CAD build for the part. Positions are in the model's coordinates, mm. Round coordinates to 2 decimals unless told otherwise and drop trailing zeros. Write each loop counter-clockwise with the first axis right and the second up, starting at its lowest first coordinate (ties: lowest second). Pieces come first, ordered by that corner, then holes. Notation, with made-up numbers: (17, 12.25) - (51, 12.25) arc R31 ccw to (51, 46.25) - close; hole circle Ø4 at (-36.5, 80.5). An arc over 180 degrees is marked (long way). Put each result on its own line as item: value. Start each with the question number.
Item 1: Cut at C-C (x = -51). Give the cut face in (y, z), and give its area (3 significant figures).
Item 2: Cut at A-A (z = 0.95). Count the separate pieces of the cut face and the enclosed holes in it, and give its area (3 significant figures).
Item 3: Pin check, flat tips, straight feed: pin 1 Ø2.5 at (x, y) = (-26.62, -9.74) entering from +Z; pin 2 Ø1.5 at (y, z) = (-11.5, 1.5) entering from -X; pin 3 Ø1.5 at (x, z) = (42.5, 1) entering from +Y; pin 4 Ø1.5 at (x, z) = (25.5, 1) entering from -Y. Stop position of each tip, or through.
Item 4: Drill centre lines: line 1 (X direction, y = -13, z = 2.85); line 2 (Y direction, x = 41.5, z = 0.6); line 3 (Y direction, x = -22.5, z = 0.55). Where is each one in solid material? Low to high. Write a range as from..to.
Item 5: Cut at B-B (x = 39.5). Give the cut face in (y, z).
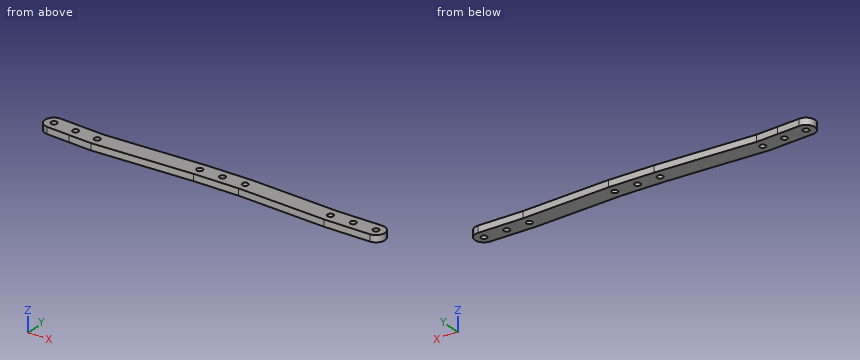
```python
from build123d import *

# Parameters (mm, degrees)
SKETCH3_R           = 1.3
SKETCH3_R_2         = 1.299999997
SKETCH3_R_3         = 1.299999994
SKETCH3_R_4         = 1.299999992
BOSS_EXTRUDE4_DEPTH = 3


with BuildPart() as part:
    # Sketch3 → Boss-Extrude4 (new body)
    with BuildSketch(Plane.XY):
        with BuildLine():
            Line((52.490961286, -7.932397294), (42.490961286, -7.932397294))
            Line((42.490961286, -7.932397294), (32.603090799, -7.932397294))
            Line((32.603090799, -7.932397294), (-6.503485734, -5.738172333))
            Line((-6.503485734, -5.738172333), (-16.615615248, -5.738172333))
            Line((-16.615615248, -5.738172333), (-26.685781884, -5.738172333))
            Line((-26.685781884, -5.738172333), (-70.669528111, -7.281743071))
            Line((-70.669528111, -7.281743071), (-80.441339321, -6.619135373))
            Line((-80.441339321, -6.619135373), (-90.418428622, -5.942608164))
            ThreePointArc((-90.418428622, -5.942608164), (-94.679875227, -9.662833001), (-90.95965039, -13.924279606))
            Line((-90.95965039, -13.924279606), (-80.982561088, -14.600806815))
            Line((-80.982561088, -14.600806815), (-70.800193694, -15.291253536))
            Line((-70.800193694, -15.291253536), (-26.545448611, -13.738172333))
            Line((-26.545448611, -13.738172333), (-16.615615248, -13.738172333))
            Line((-16.615615248, -13.738172333), (-6.727744762, -13.738172333))
            Line((-6.727744762, -13.738172333), (32.378831772, -15.932397294))
            Line((32.378831772, -15.932397294), (42.490961286, -15.932397294))
            Line((42.490961286, -15.932397294), (52.490961286, -15.932397294))
            ThreePointArc((52.490961286, -15.932397294), (56.490961286, -11.932397294), (52.490961286, -7.932397294))
        make_face()
        with Locations((-90.689039506, -9.933443885)):
            Circle(SKETCH3_R, mode=Mode.SUBTRACT)
        with Locations((-70.734860903, -11.286498303)):
            Circle(SKETCH3_R, mode=Mode.SUBTRACT)
        with Locations((-80.711950204, -10.609971094)):
            Circle(SKETCH3_R, mode=Mode.SUBTRACT)
        with Locations((-26.615615248, -9.738172333)):
            Circle(SKETCH3_R, mode=Mode.SUBTRACT)
        with Locations((-16.615615248, -9.738172333)):
            Circle(SKETCH3_R_2, mode=Mode.SUBTRACT)
        with Locations((-6.615615248, -9.738172333)):
            Circle(SKETCH3_R_3, mode=Mode.SUBTRACT)
        with Locations((32.490961286, -11.932397294)):
            Circle(SKETCH3_R_3, mode=Mode.SUBTRACT)
        with Locations((42.490961286, -11.932397294)):
            Circle(SKETCH3_R_4, mode=Mode.SUBTRACT)
        with Locations((52.490961286, -11.932397294)):
            Circle(SKETCH3_R, mode=Mode.SUBTRACT)
    extrude(amount=BOSS_EXTRUDE4_DEPTH)


solid = part.part
```
Output values:
1. outline: (-14.6, 0) - (-6.59, 0) - (-6.59, 3) - (-14.6, 3) - close
1. area: 24.0 mm2
2. separate pieces: 1
2. enclosed holes: 9
2. area: 1,150 mm2
3. pin 1: through
3. pin 2: x = -94.6
3. pin 3: y = -7.93
3. pin 4: y = -15.59
4. line 1: -93.26..31.75, 33.23..41.75, 43.23..51.75, 53.23..56.35
4. line 2: -15.93..-12.77, -11.09..-7.93
4. line 3: -13.74..-5.74
5. outline: (-15.93, 0) - (-7.93, 0) - (-7.93, 3) - (-15.93, 3) - close
